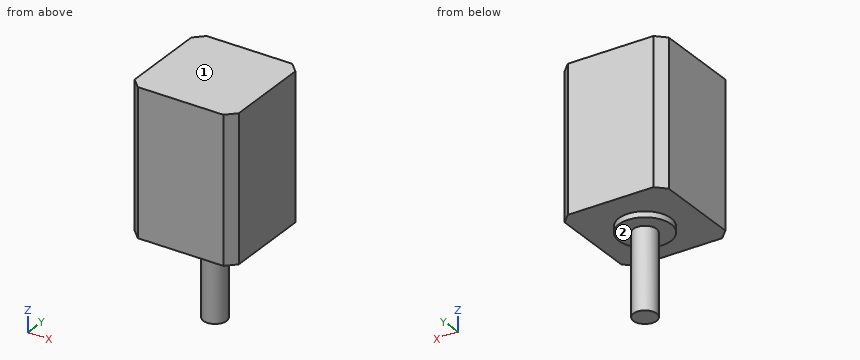
from build123d import *

# Parameters (mm, degrees)
SKETCH1_R           = 20
BOSS_EXTRUDE1_DEPTH = 140
SKETCH2_R           = 45
BOSS_EXTRUDE2_DEPTH = 10
SKETCH3_W           = 180
SKETCH3_H           = 180
BOSS_EXTRUDE3_DEPTH = 250
CHAMFER1_SIZE       = 16


with BuildPart() as part:
    # Sketch1 → Boss-Extrude1 (new body)
    with BuildSketch(Plane.XY):
        Circle(SKETCH1_R)
    extrude(amount=BOSS_EXTRUDE1_DEPTH)

    # Sketch2 → Boss-Extrude2 (add)
    with BuildSketch(Plane.XY.offset(140)):
        Circle(SKETCH2_R)
    extrude(amount=BOSS_EXTRUDE2_DEPTH)

    # Sketch3 → Boss-Extrude3 (add)
    with BuildSketch(Plane.XY.offset(150)):
        Rectangle(SKETCH3_W, SKETCH3_H)
    extrude(amount=BOSS_EXTRUDE3_DEPTH)

    # Chamfer1
    chamfer1_edges = [part.edges().sort_by_distance(p)[0] for p in [
        (90, -90, 275),
        (90, 90, 275),
        (-90, 90, 275),
        (-90, -90, 275),
    ]]
    chamfer(chamfer1_edges, length=CHAMFER1_SIZE)


solid = part.part
Read the model definition and answer for the solid it produces. Units are mm, in the model's axes. Face numbers are marked on the shaded views. A direction names the side the tool comes from. Give positions to 0.01 mm unless a question says otherwise; leave off trailing zeros. Loops run counter-clockwise (first coordinate to the right, second up) from the corner with the lowest first, then second, coordinate; pieces in that order, holes last. Notation, with made-up numbers: M 42.5,-1 L 76.5,-1 A26 ccw 76.5,20 Z; hole C -5.5,-6.75 d11. An arc over 180 degrees is marked long. Write each question's results on one line, items separated by ' | '.
1. A tool of negligible diameter and unlimited length cuts with its end or side. For the marked faces 1 and 2, from which of +Z, -Z, +X, -X, +Y, -Y can it reach the whole face along a straight path? Write none if from no direction.
Values:
face 1: +Z, +X, -X, +Y, -Y | face 2: -Z
2. Straight lines are drawn through the part: line 1 (Z direction, x = -60, y = 30); line 2 (Z direction, x = -39.5, y = -20). For each, find the intervals that lie inside material, in ascending order. Write a range as [from, to].
Values:
line 1: z = [150, 400] | line 2: z = [140, 400]
3. Section D-D on y = -36 is taken. Give the vertices of the cut face in (x, z).
Values:
outline: M -90,150 L -27,150 L -27,140 L 27,140 L 27,150 L 90,150 L 90,400 L -90,400 Z
4. Section A-A on z = 365.5 is taken. Give the vertices of the cut face in (x, y).
Values:
outline: M -90,-74 L -74,-90 L 74,-90 L 90,-74 L 90,74 L 74,90 L -74,90 L -90,74 Z
5. Given pin 1 (2 mm diameter, centred on x = -29.5, y = 49.5, fed in from -Z); pin 2 (1.5 mm diameter, centred on y = 33, z = 149, fed in from -X), each flat-ended and moving along its own axis, determine where each tip first touches the part or whether it passes through.
Values:
pin 1: stops at z = 150 | pin 2: stops at x = -31.38
6. Section B-B on y = 0 is taken. Give the vertices of the cut face in (x, z).
Values:
outline: M -90,150 L -45,150 L -45,140 L -20,140 L -20,0 L 20,0 L 20,140 L 45,140 L 45,150 L 90,150 L 90,400 L -90,400 Z
